Design review of the part shown in the three views and the two pictorial views. Dimensions are in mm from the part's minimum x, y and z. Give positions to 0.01 mm unless a question says otherwise; leave off trailing zeros. Write each loop counter-clockwise with the first axis right and the second up, starting at its lowest first coordinate (ties: lowest second). Pieces come first, ordered by that corner, then holes. Notation, with made-up numbers: M 25,48.25 L 42,48.25 A27 ccw 42,67.25 Z; hole C 38,-3.75 d10. An arc over 180 degrees is marked long. Use one line per item in the form item = value. Start each with the question number.
Q1. Consider section D-D on z = 76.5. Write out the cut boundary in (x, y), and give its area (3 significant figures).
Q2. Consider section C-C on x = 37.5. Write out the cut boundary in (y, z), and give its area (3 significant figures).
Q3. Mouldability with a two-part tool opening along Y and no side actions: class the marked faces 1 and 2 as released by +Y, released by -Y, zero draft, split by the parting line, or undercut.
Q4. Consider section A-A on y = 7. Write out the cut boundary in (x, z), and give its area (3 significant figures).
Q5. Consider section B-B on z = 32. Write out the cut boundary in (x, y), and give its area (3 significant figures).
Q6. Clearance check with flat-ended pins moving along their axes: pin 1 Ø10 at (y, z) = (24, 56) entering from +X; pin 2 Ø4 at (y, z) = (30, 17) entering from +X; pin 3 Ø1.5 at (x, z) = (13.5, 66) entering from -Y; pin 4 Ø22.5 at (x, y) = (43, 30.5) entering from +Z. State where each tip first meets the part, or that it passes through.
Q7. For probe 1 along X at (y, z) = (22.5, 33.5); probe 2 along Z at (x, y) = (19, 19.5) (1 decimal); probe 3 along Z at (x, y) = (33.5, 39.5), list the stretches that pass through material, from the lowest coordinate up. Write a range as [from, to].
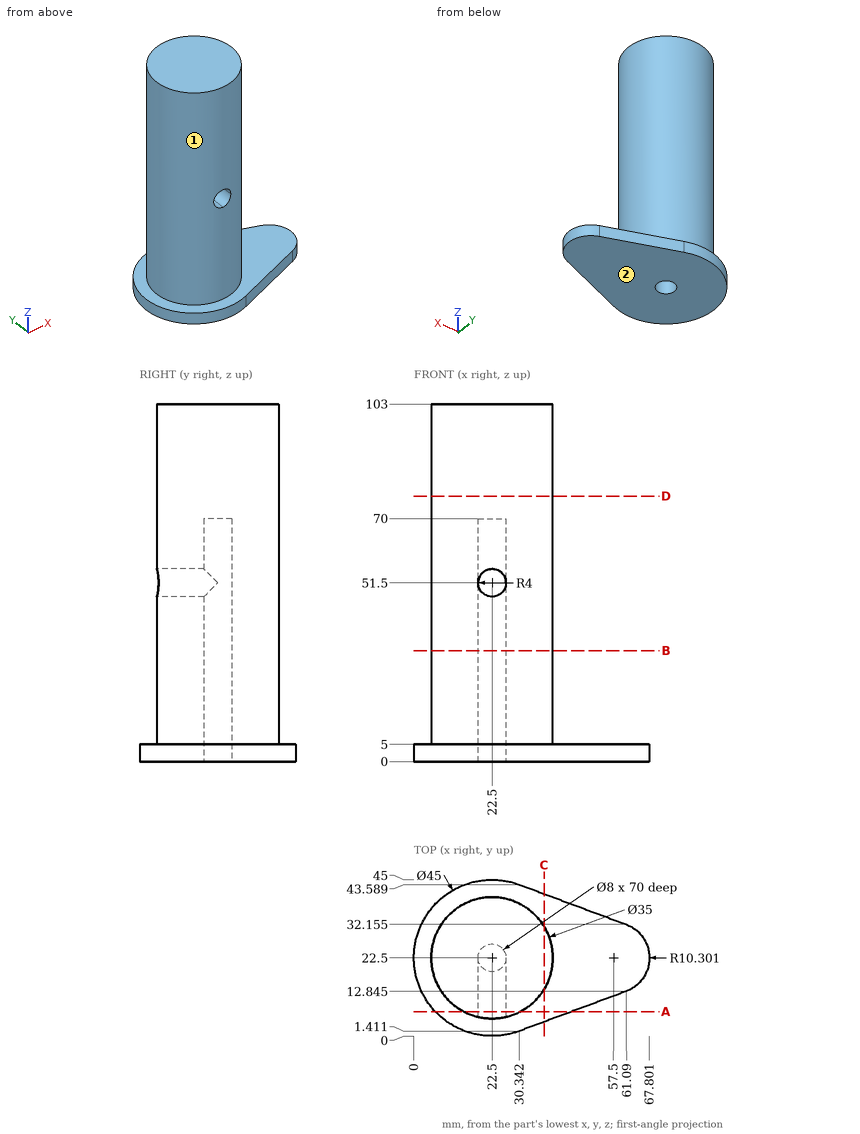
Working result:
q1.outline = C 22.5,22.5 d35
q1.area = 962 mm²
q2.outline = M 4.07,0 L 40.93,0 L 40.93,5 L 31.51,5 L 31.51,103 L 13.49,103 L 13.49,5 L 4.07,5 Z
q2.area = 1,950 mm²
q3.face_1 = split by the parting line
q3.face_2 = zero draft
q4.outline = M 6.19,0 L 45.37,0 L 45.37,5 L 30.62,5 L 30.62,103 L 14.38,103 L 14.38,5 L 6.19,5 Z; hole C 22.5,51.5 d8
q4.area = 1,740 mm²
q5.outline = C 22.5,22.5 d35; hole C 22.5,22.5 d8
q5.area = 912 mm²
q6.pin_1 = 40
q6.pin_2 = 39.11
q6.pin_3 = 7.07
q6.pin_4 = 103
q7.probe_1 = [5, 18.5], [26.5, 40]
q7.probe_2 = [0, 49.6], [53.4, 103]
q7.probe_3 = [0, 5]
